Check sheet for the modelled part. Datum: model origin and axes. Units: mm. Face numbers are marked on the shaded views. A direction names the side the tool comes from. Round coordinates to 2 decimals unless told otherwise and drop trailing zeros. Write each loop counter-clockwise with the first axis right and the second up, starting at its lowest first coordinate (ties: lowest second). Pieces come first, ordered by that corner, then holes. Notation, with made-up numbers: M 53.5,-8 L 64.5,-8 A18 cw 64.5,12 Z; hole C 42.5,-6 d10. An arc over 180 degrees is marked long. Answer in a Markdown table with one row per item.
```python
from build123d import *

# Parameters (mm, degrees)
SKETCH_1_W                = 95
SKETCH_1_H                = 63
EXTRUDE_1_DEPTH           = 12
SKETCH_9_W                = 15.5
SKETCH_9_H                = 51
CUT_EXTRUDE_4_DEPTH       = 115.621114983
HOLE_WIZARD_6_5_6_5_1_D   = 4.5
SKETCH_12_R               = 17.5
CUT_EXTRUDE_5_DEPTH       = 115.621114983
FILLET_1_R                = 10
HOLE_WIZARD_5_0_5_1_D     = 5
HOLE_WIZARD_5_0_5_1_DEPTH = 10
HOLE_WIZARD_5_0_5_1_TIP   = 1.502151548
FILLET_2_R                = 2
HOLE_WIZARD_1_D           = 6.4
HOLE_WIZARD_1_CBORE_D     = 11
HOLE_WIZARD_1_CBORE_DEPTH = 7


with BuildPart() as part:
    # 草图1 → 凸台-拉伸1 (new body)
    with BuildSketch(Plane(origin=(0, 0, 0), x_dir=(1, 0, 0), z_dir=(0, 1, 0))):
        with Locations((47.5, -31.5)):
            Rectangle(SKETCH_1_W, SKETCH_1_H)
    extrude(amount=EXTRUDE_1_DEPTH)

    # 草图9 → 切除-拉伸4 (cut, through all)
    with BuildSketch(Plane(origin=(0, 12, 0), x_dir=(1, 0, 0), z_dir=(0, 1, 0))):
        with Locations((7.75, -37.5)):
            Rectangle(SKETCH_9_W, SKETCH_9_H)
        with Locations((87.25, -37.5)):
            Rectangle(SKETCH_9_W, SKETCH_9_H)
    extrude(amount=-CUT_EXTRUDE_4_DEPTH, mode=Mode.SUBTRACT)

    # Ø6.5 (6.5) 直径孔1 (through all)
    with Locations(Plane.XY.offset(12)):
        with Locations((6, 6), (89, 6)):
            Hole(HOLE_WIZARD_6_5_6_5_1_D / 2)

    # 草图12 → 切除-拉伸5 (cut, through all)
    with BuildSketch(Plane(origin=(0, 12, 0), x_dir=(1, 0, 0), z_dir=(0, 1, 0))):
        with Locations(Location((47.5, -36.5, 0), (0, 0, 270))):
            Circle(SKETCH_12_R)
    extrude(amount=-CUT_EXTRUDE_5_DEPTH, mode=Mode.SUBTRACT)

    # 圆角1
    fillet_1_edges = [part.edges().sort_by_distance(p)[0] for p in [
        (15.5, 6, 63),
        (79.5, 6, 63),
    ]]
    fillet(fillet_1_edges, radius=FILLET_1_R)

    # Ø5.0 (5) 直径孔1
    with Locations(Plane(origin=(0, 0, 0), x_dir=(-1, 0, 0), z_dir=(0, 0, -1))):
        with Locations((-67.5, 6), (-27.5, 6)):
            Hole(HOLE_WIZARD_5_0_5_1_D / 2, depth=HOLE_WIZARD_5_0_5_1_DEPTH)
            with Locations((0, 0, -(HOLE_WIZARD_5_0_5_1_DEPTH + HOLE_WIZARD_5_0_5_1_TIP / 2))):  # 118° drill point
                Cone(0, HOLE_WIZARD_5_0_5_1_D / 2, HOLE_WIZARD_5_0_5_1_TIP, mode=Mode.SUBTRACT)

    # 圆角2
    fillet_2_edges = [part.edges().sort_by_distance(p)[0] for p in [
        (15.5, 6, 12),
        (79.5, 6, 12),
    ]]
    fillet(fillet_2_edges, radius=FILLET_2_R)

    # 打孔尺寸(%根据)内六角圆柱头螺钉的类型1 (through all)
    with Locations(Plane(origin=(0, 0, 0), x_dir=(-1, 0, 0), z_dir=(0, -1, 0))):
        with Locations((-67.5, -56.5), (-27.5, -56.5), (-27.5, -16.5), (-67.5, -16.5)):
            CounterBoreHole(HOLE_WIZARD_1_D / 2, HOLE_WIZARD_1_CBORE_D / 2, HOLE_WIZARD_1_CBORE_DEPTH)


solid = part.part
```
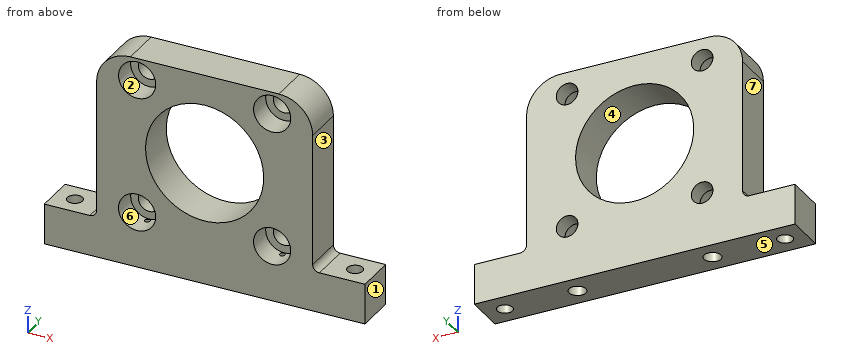
1. Section check D-D, the plane z = 6. Record the cut outline in (x, y).
Found:
| item | result |
|---|---|
| outline | M 0,0 L 95,0 L 95,12 L 0,12 Z; hole C 6,6 d4.5; hole C 27.5,6 d5; hole C 67.5,6 d5; hole C 89,6 d4.5 |
2. Draft check along Z on the marked faces 4, 5, 6 and 7. Enter one of: +Z half, -Z half, draft (parallel to the pull), parting line (faces both ways), or undercut.
Found:
| item | result |
|---|---|
| face 4 | undercut |
| face 5 | -Z half |
| face 6 | undercut |
| face 7 | draft |
3. Access from +Z, -Z, +X, -X, +Y, -Y to the whole of each face (thin tool, end or side, straight path). Record for the marked faces 1, 2 and 3.
Found:
| item | result |
|---|---|
| face 1 | +Z, -Z, +X, +Y, -Y |
| face 2 | -Y |
| face 3 | +Z, +X, +Y, -Y |
4. Section check C-C, the plane x = 6. Record the cut outline in (y, z), and give its area (3 significant figures).
Found:
| item | result |
|---|---|
| outline | M 0,0 L 3.75,0 L 3.75,12 L 0,12 Z; M 8.25,0 L 12,0 L 12,12 L 8.25,12 Z |
| area | 90.0 mm2 |
5. Scan lines: L1, parallel to Z at x = 27.5, y = 2.25; L2, parallel to Z at x = 27.5, y = 10.5; L3, parallel to X at y = 3.25, z = 16.5. Record each from-to range of solid material in increasing order.
Found:
| item | result |
|---|---|
| L1 | z = 0 to 11, 22 to 51, 62 to 63 |
| L2 | z = 0 to 13.3, 19.7 to 53.3, 59.7 to 63 |
| L3 | x = 15.5 to 22, 33 to 62, 73 to 79.5 |
6. Section check B-B, the plane y = 9.75. Record the cut outline in (x, z), and give its area (3 significant figures).
Found:
| item | result |
|---|---|
| outline | M 0,0 L 95,0 L 95,12 L 81.5,12 A2 cw 79.5,14 L 79.5,53 A10 ccw 69.5,63 L 25.5,63 A10 ccw 15.5,53 L 15.5,14 A2 cw 13.5,12 L 0,12 Z; hole C 27.5,16.5 d6.4; hole C 27.5,56.5 d6.4; hole C 47.5,36.5 d35; hole C 67.5,16.5 d6.4; hole C 67.5,56.5 d6.4 |
| area | 3,270 mm2 |
7. Go/stop test with flat-tipped pins: pin 1 (3.5 mm diameter, centred on y = 3.5, z = 24.5, fed in from +X); pin 2 (3 mm diameter, centred on x = 67.5, y = 6, fed in from -Z); pin 3 (3.5 mm diameter, centred on x = 65.5, z = 18, fed in from -Y). Record where each tip stops, or that it passes through.
Found:
| item | result |
|---|---|
| pin 1 | stops at x = 79.5 |
| pin 2 | stops at z = 10.6 |
| pin 3 | stops at y = 7 |
8. Section check A-A, the plane z = 16.5. Record the cut outline in (x, y).
Found:
| item | result |
|---|---|
| outline | M 15.5,0 L 22,0 L 22,7 L 24.3,7 L 24.3,12 L 15.5,12 Z; M 30.7,7 L 33,7 L 33,0 L 62,0 L 62,7 L 64.3,7 L 64.3,12 L 30.7,12 Z; M 70.7,7 L 73,7 L 73,0 L 79.5,0 L 79.5,12 L 70.7,12 Z |
